```python
from build123d import *

# Parameters (mm, degrees)
SKETCH1_W           = 80
SKETCH1_H           = 26
BOSS_EXTRUDE1_DEPTH = 9
CUT_EXTRUDE1_REACH  = 45.012
SKETCH2_R           = 2.6
SKETCH3_R           = 4.5
CUT_EXTRUDE2_DEPTH  = 5.2
CUT_EXTRUDE3_REACH  = 45.012
SKETCH8_W           = 62.5
SKETCH8_H           = 26
CUT_EXTRUDE5_DEPTH  = 1
CHAMFER1_SIZE       = 1


with BuildPart() as part:
    # Sketch1 → Boss-Extrude1 (new body)
    with BuildSketch(Plane.XY):
        Rectangle(SKETCH1_W, SKETCH1_H)
    extrude(amount=BOSS_EXTRUDE1_DEPTH)

    # Sketch2 → Cut-Extrude1 (cut, up to next)
    with BuildSketch(Plane.XY.offset(9), mode=Mode.PRIVATE) as cut_extrude1_sk1:
        with Locations((-27, -8)):
            Circle(SKETCH2_R)
    cut_extrude1_tool1 = extrude(cut_extrude1_sk1.sketch, amount=-CUT_EXTRUDE1_REACH, mode=Mode.PRIVATE) & part.part
    # Sketch2 → Cut-Extrude1 (cut, up to next)
    with BuildSketch(Plane.XY.offset(9), mode=Mode.PRIVATE) as cut_extrude1_sk2:
        with Locations((-27, 8)):
            Circle(SKETCH2_R)
    cut_extrude1_tool2 = extrude(cut_extrude1_sk2.sketch, amount=-CUT_EXTRUDE1_REACH, mode=Mode.PRIVATE) & part.part
    # Sketch2 → Cut-Extrude1 (cut, up to next)
    with BuildSketch(Plane.XY.offset(9), mode=Mode.PRIVATE) as cut_extrude1_sk3:
        with Locations((27, 8)):
            Circle(SKETCH2_R)
    cut_extrude1_tool3 = extrude(cut_extrude1_sk3.sketch, amount=-CUT_EXTRUDE1_REACH, mode=Mode.PRIVATE) & part.part
    # Sketch2 → Cut-Extrude1 (cut, up to next)
    with BuildSketch(Plane.XY.offset(9), mode=Mode.PRIVATE) as cut_extrude1_sk4:
        with Locations((27, -8)):
            Circle(SKETCH2_R)
    cut_extrude1_tool4 = extrude(cut_extrude1_sk4.sketch, amount=-CUT_EXTRUDE1_REACH, mode=Mode.PRIVATE) & part.part
    add(cut_extrude1_tool1.solids().sort_by_distance((-27, -8, 9))[0], mode=Mode.SUBTRACT)
    add(cut_extrude1_tool2.solids().sort_by_distance((-27, 8, 9))[0], mode=Mode.SUBTRACT)
    add(cut_extrude1_tool3.solids().sort_by_distance((27, 8, 9))[0], mode=Mode.SUBTRACT)
    add(cut_extrude1_tool4.solids().sort_by_distance((27, -8, 9))[0], mode=Mode.SUBTRACT)

    # Sketch3 → Cut-Extrude2 (cut)
    with BuildSketch(Plane.XY.offset(9)):
        with Locations((-27, -8)):
            Circle(SKETCH3_R)
        with Locations((-27, 8)):
            Circle(SKETCH3_R)
        with Locations((27, 8)):
            Circle(SKETCH3_R)
        with Locations((27, -8)):
            Circle(SKETCH3_R)
    extrude(amount=-CUT_EXTRUDE2_DEPTH, mode=Mode.SUBTRACT)

    # Sketch6 → Cut-Extrude3 (cut, up to next)
    with BuildSketch(Plane(origin=(0, 0, 0), x_dir=(-1, 0, 0), z_dir=(0, 0, -1)), mode=Mode.PRIVATE) as cut_extrude3_sk1:
        with BuildLine():
            Line((-33.25, 8.5), (-33.25, -8.5))
            ThreePointArc((-33.25, -8.5), (-35.5, -10.75), (-37.75, -8.5))
            Line((-37.75, -8.5), (-37.75, 8.5))
            ThreePointArc((-37.75, 8.5), (-35.5, 10.75), (-33.25, 8.5))
        make_face()
    cut_extrude3_tool1 = extrude(cut_extrude3_sk1.sketch, amount=-CUT_EXTRUDE3_REACH, mode=Mode.PRIVATE) & part.part
    cut_extrude3 = cut_extrude3_tool1.solids().sort_by_distance((35.5, 0, 0))[0]
    add(cut_extrude3, mode=Mode.SUBTRACT)

    # Mirror1: Cut-Extrude3 across plane
    add(cut_extrude3.mirror(Plane(origin=(0, 0, 0), x_dir=(0, 0, 1), z_dir=(1, 0, 0))), mode=Mode.SUBTRACT)

    # Sketch8 → Cut-Extrude5 (cut)
    with BuildSketch(Plane(origin=(0, 0, 0), x_dir=(-1, 0, 0), z_dir=(0, 0, -1))):
        Rectangle(SKETCH8_W, SKETCH8_H)
    extrude(amount=-CUT_EXTRUDE5_DEPTH, mode=Mode.SUBTRACT)

    # Chamfer1
    chamfer1_edges = [part.edges().sort_by_distance(p)[0] for p in [
        (40, -13, 4.5),
        (-40, -13, 4.5),
        (-40, 13, 4.5),
        (40, 13, 4.5),
    ]]
    chamfer(chamfer1_edges, length=CHAMFER1_SIZE)


solid = part.part
```
Work out the finished part from the listing and answer in its coordinate system (mm). A direction names the side the tool comes from. Round coordinates to 2 decimals unless told otherwise and drop trailing zeros. Write each loop counter-clockwise with the first axis right and the second up, starting at its lowest first coordinate (ties: lowest second). Pieces come first, ordered by that corner, then holes.
1) Which of the six approach directions +Z, -Z, +X, -X, +Y, -Y give full straight-line access (tool end or side, diameter ignored) to faces 3 (the face through (0, 0, 1)), 4 (the face through (-1, 0, 9)), 5 (the face through (-25, -10, 3.8)), 6 (the face through (35.45, -10.75, 4.44))?
2) A cutting plane is placed at C-C on z = 5. Determine the outline of the cut face in (x, y), and give its area (3 significant figures).
3) A cutting plane is placed at D-D on y = -9.25. Give the number of separate pieces and of enclosed holes in the cut face, and give its area (3 significant figures).
4) A cutting plane is placed at B-B on x = -35.5. Determine the outline of the cut face in (y, z), and give its area (3 significant figures).
5) Determine the mould class of faces 1 (the face through (-37.75, 0, 4)), 2 (the face through (-1, 13, 4)) for opening direction X: pulls with the +X half, pulls with the -X half, needs draft (parallel to the pull), parting line crosses it, or undercut.
6) A cutting plane is placed at A-A on x = -27. Determine the outline of the cut face in (y, z), and give its area (3 significant figures).
7) Consider probe 1 along X at (y, z) = (0, 7.5); probe 2 along Y at (x, z) = (-27, 2.6); probe 3 along Y at (x, z) = (-27, 4.9). Determine where each line is inside the solid, lowest interval first.
8) Flat-ended cylindrical pins translate along their axes: P1, Ø2, axis at x = -19, y = -3, coming from the -Z side; P2, Ø6, axis at x = -27, y = -8, coming from the +Z side; P3, Ø4.5, axis at x = -27, y = 8, coming from the +Z side. Find the tip coordinate at first contact, or state that the pin passes through.
Entries:
1. face 3: -Z, +Y, -Y
1. face 4: +Z, +X, -X, +Y, -Y
1. face 5: +Z
1. face 6: +Z, -Z
2. outline: (-40, -12) - (-39, -13) - (39, -13) - (40, -12) - (40, 12) - (39, 13) - (-39, 13) - (-40, 12) - close; hole (-37.75, -8.5) arc R2.25 ccw to (-33.25, -8.5) - (-33.25, 8.5) arc R2.25 ccw to (-37.75, 8.5) - close; hole circle Ø9 at (-27, -8); hole circle Ø9 at (-27, 8); hole circle Ø9 at (27, -8); hole circle Ø9 at (27, 8); hole (33.25, -8.5) arc R2.25 ccw to (37.75, -8.5) - (37.75, 8.5) arc R2.25 ccw to (33.25, 8.5) - close
2. area: 1,640 mm2
3. separate pieces: 5
3. enclosed holes: 0
3. area: 466 mm2
4. outline: (-13, 0) - (-10.75, 0) - (-10.75, 9) - (-13, 9) - close; (10.75, 0) - (13, 0) - (13, 9) - (10.75, 9) - close
4. area: 40.5 mm2
5. face 1: undercut
5. face 2: needs draft
6. outline: (-13, 1) - (-10.6, 1) - (-10.6, 3.8) - (-12.5, 3.8) - (-12.5, 9) - (-13, 9) - close; (-5.4, 1) - (5.4, 1) - (5.4, 3.8) - (3.5, 3.8) - (3.5, 9) - (-3.5, 9) - (-3.5, 3.8) - (-5.4, 3.8) - close; (10.6, 1) - (13, 1) - (13, 9) - (12.5, 9) - (12.5, 3.8) - (10.6, 3.8) - close
6. area: 85.3 mm2
7. probe 1: x = -40 to -37.75, -33.25 to 33.25, 37.75 to 40
7. probe 2: y = -13 to -10.6, -5.4 to 5.4, 10.6 to 13
7. probe 3: y = -13 to -12.5, -3.5 to 3.5, 12.5 to 13
8. P1: stops at z = 1
8. P2: stops at z = 3.8
8. P3: passes through
